Check sheet for the modelled part. Datum: model origin and axes. Units: mm. Round coordinates to 2 decimals unless told otherwise and drop trailing zeros. Order: outer loops, then holes, each group sorted by start corner. A loop starts at its lowest first (then second) coordinate and runs counter-clockwise, first axis right, second up. Notation, with made-up numbers: (-31.5, -6) -> (-18.5, -6) arc R5 ccw to (-18.5, 2) -> close; hole circle Ø3 at (31, 24). An arc over 180 degrees is marked (long way). Answer in a Markdown table with one row per item.
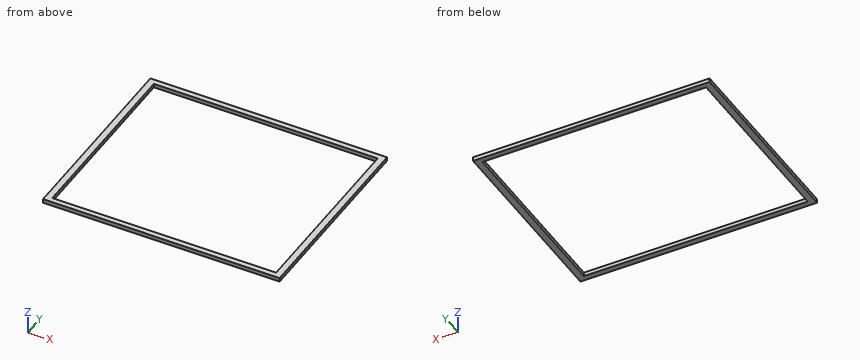
from build123d import *

# Parameters (mm, degrees)
SKETCH1_W           = 600
SKETCH1_H           = 500
SKETCH1_W_2         = 567.390239782
SKETCH1_H_2         = 472.825199818
BOSS_EXTRUDE1_DEPTH = 10


with BuildPart() as part:
    # Sketch1 → Boss-Extrude1 (new body)
    with BuildSketch(Plane.XY):
        Rectangle(SKETCH1_W, SKETCH1_H)
        Rectangle(SKETCH1_W_2, SKETCH1_H_2, mode=Mode.SUBTRACT)
    extrude(amount=BOSS_EXTRUDE1_DEPTH)


solid = part.part
Item 1: Cross-section at A-A (y = -18). Record the boundary of the cut face in (x, z), and give its area (3 significant figures).
Result sheet:
| item | result |
|---|---|
| outline | (-300, 0) -> (-283.7, 0) -> (-283.7, 10) -> (-300, 10) -> close; (283.7, 0) -> (300, 0) -> (300, 10) -> (283.7, 10) -> close |
| area | 326 mm^2 |
Item 2: Scan lines: line 1 (Y direction, x = 30, z = 7.75); line 2 (X direction, y = -114, z = 5.25). Record each from-to range of solid material in increasing order. Write a range as [from, to].
Result sheet:
| item | result |
|---|---|
| line 1 | y = [-250, -236.41], [236.41, 250] |
| line 2 | x = [-300, -283.7], [283.7, 300] |
Item 3: Cross-section at C-C (z = 4.5). Record the boundary of the cut face in (x, y).
Result sheet:
| item | result |
|---|---|
| outline | (-300, -250) -> (300, -250) -> (300, 250) -> (-300, 250) -> close; hole (-283.7, -236.41) -> (283.7, -236.41) -> (283.7, 236.41) -> (-283.7, 236.41) -> close |
Item 4: Cross-section at B-B (x = 246). Record the boundary of the cut face in (y, z), and give its area (3 significant figures).
Result sheet:
| item | result |
|---|---|
| outline | (-250, 0) -> (-236.41, 0) -> (-236.41, 10) -> (-250, 10) -> close; (236.41, 0) -> (250, 0) -> (250, 10) -> (236.41, 10) -> close |
| area | 272 mm^2 |
